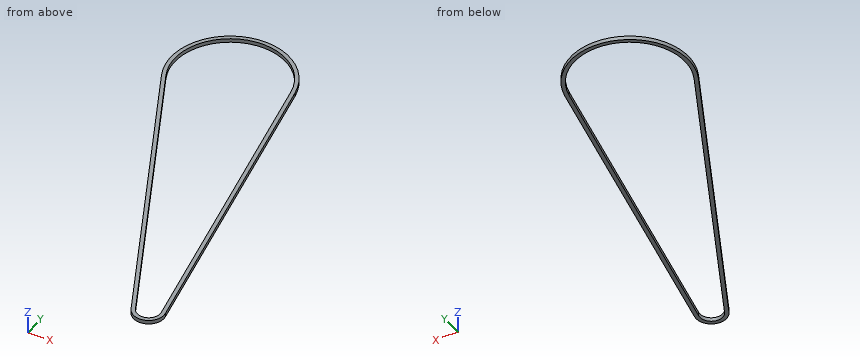
```python
from build123d import *

# Parameters (mm, degrees)
THIN_WALL_EXTRUDE1_DEPTH = 10


with BuildPart() as part:
    # Sketch1 → Thin-wall extrude1 (new body)
    with BuildSketch(Plane.XY):
        with BuildLine():
            Line((153.510023011, 111.669421793), (308.383834576, -735.55582317))
            ThreePointArc((308.383834576, -735.55582317), (281.282561977, -781.001122311), (232.629670707, -760.200873238))
            Line((232.629670707, -760.200873238), (-140.636470033, 15.974945367))
            ThreePointArc((-140.636470033, 15.974945367), (-48.278259042, 232.005723732), (153.510023011, 111.669421793))
        make_face()
        with BuildLine():
            Line((143.673030314, 109.87120749), (298.546841879, -737.354037473))
            ThreePointArc((298.546841879, -737.354037473), (278.18886899, -771.491702575), (241.641720223, -755.866941592))
            Line((241.641720223, -755.866941592), (-131.624420517, 20.308877014))
            ThreePointArc((-131.624420517, 20.308877014), (-45.184566055, 222.496303997), (143.673030314, 109.87120749))
        make_face(mode=Mode.SUBTRACT)
    extrude(amount=THIN_WALL_EXTRUDE1_DEPTH)


solid = part.part
```
Verification items for the finished model (mm, model axes). Give positions to 0.01 mm unless a question says otherwise; leave off trailing zeros. Loops run counter-clockwise (first coordinate to the right, second up) from the corner with the lowest first, then second, coordinate; pieces in that order, holes last.
1. Go/stop test with flat-tipped pins: pin 1 Ø3 at (x, z) = (50, 5) entering from -Y; pin 2 Ø2 at (x, z) = (-98, 4.5) entering from +Y; pin 3 Ø1.5 at (y, z) = (132.5, 9) entering from -X. Record where each tip stops, or that it passes through.
2. Section check B-B, the plane x = 0. Enter the section's corners in (y, z), then the cut area to 3 significant figures.
3. Section check A-A, the plane z = 4.5. Enter the section's corners in (x, y).
4. Section check C-C, the plane y = 75.5. Enter the section's corners in (x, z).
5. Thickness scan on line 1 (X direction, y = -348.5, z = 9.25); line 2 (Y direction, x = 32, z = 6.5); line 3 (X direction, y = -334.5, z = 8). Record the ranges inside material, lowest first.
Geometry says:
1. pin 1: stops at y = -383.56
1. pin 2: stops at y = 205.85
1. pin 3: stops at x = -148.44
2. outline: (-276.47, 0) - (-253.39, 0) - (-253.39, 10) - (-276.47, 10) - close; (229.66, 0) - (239.66, 0) - (239.66, 10) - (229.66, 10) - close
2. area: 331 mm2
3. outline: (-140.64, 15.97) - (232.63, -760.2) arc R40.19 ccw to (308.38, -735.56) - (153.51, 111.67) arc R156.05 ccw (long way) to start; hole (-131.62, 20.31) - (241.64, -755.87) arc R30.19 ccw to (298.55, -737.35) - (143.67, 109.87) arc R146.05 ccw (long way) to start
4. outline: (-155.84, 0) - (-145.83, 0) - (-145.83, 10) - (-155.84, 10) - close; (149.96, 0) - (160.12, 0) - (160.12, 10) - (149.96, 10) - close
5. line 1: x = 34.64 to 45.74, 227.46 to 237.63
5. line 2: y = -343.01 to -319.93, 226.11 to 236.35
5. line 3: x = 27.91 to 39, 224.9 to 235.07
